Geometry check sheet. Reference: the model listing, model coordinates, mm. Coordinates: 2 decimals unless noted, no trailing zeros. Write each loop counter-clockwise with the first axis right and the second up, starting at its lowest first coordinate (ties: lowest second). Pieces come first, ordered by that corner, then holes. Notation, with made-up numbers: (79.5, 84) - (128.5, 84) arc R18 ccw to (128.5, 105) - close; hole circle Ø8 at (75, 47). An arc over 180 degrees is marked (long way). Answer as a JSON object with one key per item and string values. Group by question number.
from build123d import *

# Parameters (mm, degrees)
SKETCH1_W             = 28
SKETCH1_H             = 8
SKETCH1_R             = 1.25
BOSS_EXTRUDE1_DEPTH   = 3
M3_TAPPED_HOLE6_D     = 2.5
M3_TAPPED_HOLE6_DEPTH = 7.5
M3_TAPPED_HOLE6_TIP   = 0.751075774
M3_TAPPED_HOLE1_D     = 2.5
M3_TAPPED_HOLE1_DEPTH = 7.5
M3_TAPPED_HOLE1_TIP   = 0.751075774


with BuildPart() as part:
    # Sketch1 → Boss-Extrude1 (new body)
    with BuildSketch(Plane.XY):
        with Locations((14, -4)):
            Rectangle(SKETCH1_W, SKETCH1_H)
        with Locations((4, -4)):
            Circle(SKETCH1_R, mode=Mode.SUBTRACT)
        with Locations(Location((24, -4, 0), (0, 0, 180))):
            Circle(SKETCH1_R, mode=Mode.SUBTRACT)
    extrude(amount=BOSS_EXTRUDE1_DEPTH)

    # M3 Tapped Hole6
    with Locations(Plane(origin=(4, -4, 3), x_dir=(1, 0, 0), z_dir=(0, 0, 1))):
        with Locations((0, 0), (20, 0)):
            Hole(M3_TAPPED_HOLE6_D / 2, depth=M3_TAPPED_HOLE6_DEPTH)
            with Locations((0, 0, -(M3_TAPPED_HOLE6_DEPTH + M3_TAPPED_HOLE6_TIP / 2))):  # 118° drill point
                Cone(0, M3_TAPPED_HOLE6_D / 2, M3_TAPPED_HOLE6_TIP, mode=Mode.SUBTRACT)

    # M3 Tapped Hole1
    with Locations(Plane(origin=(14, -4, 3), x_dir=(1, 0, 0), z_dir=(0, 0, 1))):
        with Locations((0, 0)):
            Hole(M3_TAPPED_HOLE1_D / 2, depth=M3_TAPPED_HOLE1_DEPTH)
            with Locations((0, 0, -(M3_TAPPED_HOLE1_DEPTH + M3_TAPPED_HOLE1_TIP / 2))):  # 118° drill point
                Cone(0, M3_TAPPED_HOLE1_D / 2, M3_TAPPED_HOLE1_TIP, mode=Mode.SUBTRACT)


solid = part.part
(1) Section check C-C (x = 4.5). Record the cut outline in (y, z), and give its area (3 significant figures).
(2) Section check A-A (x = 14). Record the cut outline in (y, z).
(3) Draft check along X on faces 1 (the face through (28, -4, 1)), 2 (the face through (22.845, -3.521, 1.479)), 3 (the face through (0, -4, 1)), 4 (the face through (14, -2, 0)). Enter one of: +X half, -X half, draft (parallel to the pull), parting line (faces both ways), or undercut.
(4) Section check B-B (z = 2.65). Record the cut outline in (x, y).
(5) Gauge pin test, flat ends, axial feed: pin 1 (2 mm diameter, centred on x = 4, y = -4, fed in from -Z); pin 2 (4 mm diameter, centred on x = 14, y = -4, fed in from -Z). Record the tip position at first contact, or that the pin passes through.
(6) Material ranges on L1, parallel to Y at x = 4, z = 1.65; L2, parallel to X at y = -3.5, z = 0.7; L3, parallel to X at y = -3, z = 2.3, recorded low to high. Write a range as [from, to].
Conclusion:
{
 "1": {"outline": "(-8, 0) - (-5.15, 0) - (-5.15, 3) - (-8, 3) - close; (-2.85, 0) - (0, 0) - (0, 3) - (-2.85, 3) - close", "area": "17.1 mm^2"},
 "2": {"outline": "(-8, 0) - (-5.25, 0) - (-5.25, 3) - (-8, 3) - close; (-2.75, 0) - (0, 0) - (0, 3) - (-2.75, 3) - close"},
 "3": {"face 1": "+X half", "face 2": "undercut", "face 3": "-X half", "face 4": "draft"},
 "4": {"outline": "(0, -8) - (28, -8) - (28, 0) - (0, 0) - close; hole circle Ø2.5 at (4, -4); hole circle Ø2.5 at (14, -4); hole circle Ø2.5 at (24, -4)"},
 "5": {"pin 1": "passes through", "pin 2": "stops at z = 0"},
 "6": {"L1": "y = [-8, -5.25], [-2.75, 0]", "L2": "x = [0, 2.85], [5.15, 12.85], [15.15, 22.85], [25.15, 28]", "L3": "x = [0, 3.25], [4.75, 13.25], [14.75, 23.25], [24.75, 28]"}
}
